Input: part model. Units: mm. Frame: model coordinates. Face numbers are marked on the shaded views. A direction names the side the tool comes from. Round coordinates to 2 decimals unless told otherwise and drop trailing zeros. Write each loop counter-clockwise with the first axis right and the second up, starting at its lowest first coordinate (ties: lowest second). Pieces come first, ordered by that corner, then holes. Notation, with made-up numbers: (-8.75, 73.25) - (42.25, 73.25) arc R27 cw to (42.25, 103.25) - close; hole circle Ø1 at (-37, 44). An arc over 180 degrees is marked (long way). Use one line per item in the form item = value.
```python
from build123d import *

# Parameters (mm, degrees)
EXTRUDE_1_DEPTH     = 10
SKETCH_2_R          = 2.75
CUT_EXTRUDE_1_DEPTH = 117.404467268


with BuildPart() as part:
    # 草图1 → 凸台-拉伸1 (new body)
    with BuildSketch(Plane.XY):
        Polygon((0, 0), (0, -110), (15, -110), (15, -115), (-8, -115), (-8, 0), align=None)
    extrude(amount=EXTRUDE_1_DEPTH)

    # 草图2 → 切除-拉伸1 (cut, through all)
    with BuildSketch(Plane.XZ.offset(115)):
        with Locations(Location((6.5, 5, 0), (0, 0, 270))):
            Circle(SKETCH_2_R)
    extrude(amount=-CUT_EXTRUDE_1_DEPTH, mode=Mode.SUBTRACT)


solid = part.part
```
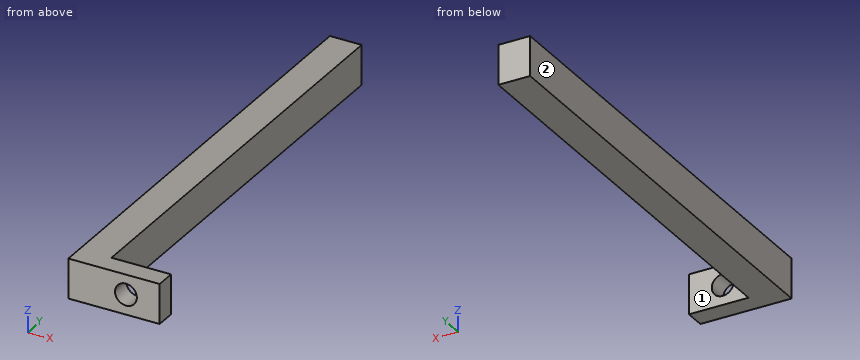
(1) Cut plane D-D on x = 11.5. Output: boundary loops of the cut face in (y, z), then the cut area to 3 significant figures.
Derived:
outline = (-115, 0) - (-110, 0) - (-110, 10) - (-115, 10) - close
area = 50.0 mm^2
(2) First-contact query: pin 1 Ø3 at (x, z) = (5, 4.5) entering from +Y; pin 2 Ø4 at (x, z) = (-4, 4.5) entering from +Y; pin 3 Ø5 at (y, z) = (-36, 2) entering from +X. Flat tips, straight axial feed; report the tip coordinate or a pass-through.
Derived:
pin_1 = -110
pin_2 = 0
pin_3 = 0
(3) Cut plane A-A on z = 5. Output: boundary loops of the cut face in (x, y).
Derived:
outline = (-8, -115) - (3.75, -115) - (3.75, -110) - (0, -110) - (0, 0) - (-8, 0) - close; (9.25, -115) - (15, -115) - (15, -110) - (9.25, -110) - close
(4) Cut plane C-C on y = -13. Output: boundary loops of the cut face in (x, z), then the cut area to 3 significant figures.
Derived:
outline = (-8, 0) - (0, 0) - (0, 10) - (-8, 10) - close
area = 80.0 mm^2
(5) Material intervals for L1, parallel to X at y = -111.8, z = 5; L2, parallel to X at y = -84, z = 1.5; L3, parallel to Y at x = 2.5, z = 2.25, sorted ascending.
Derived:
L1 = -8 to 3.75, 9.25 to 15
L2 = -8 to 0
L3 = -115 to -110
(6) Access query for the marked faces 1 and 2. Directions: +Z, -Z, +X, -X, +Y, -Y. A direction counts if a zero-diameter tool reaches every point of the face in a straight line with its end or side. Return the directions, or none.
Derived:
face_1 = +Z, -Z, +X, +Y
face_2 = +Z, -Z, -X, +Y, -Y
(7) Cut plane B-B on x = 6.5. Output: boundary loops of the cut face in (y, z), then the cut area to 3 significant figures.
Derived:
outline = (-115, 0) - (-110, 0) - (-110, 2.25) - (-115, 2.25) - close; (-115, 7.75) - (-110, 7.75) - (-110, 10) - (-115, 10) - close
area = 22.5 mm^2
